The model under review builds one solid part; all positions refer to its coordinate system, in mm. A direction names the side the tool comes from. Give positions to 0.01 mm unless a question says otherwise; leave off trailing zeros. Loops run counter-clockwise (first coordinate to the right, second up) from the corner with the lowest first, then second, coordinate; pieces in that order, holes last. Notation, with made-up numbers: (70.25, -24.75) -> (74.25, -24.75) arc R11 ccw to (74.25, -5.75) -> close; hole circle Ø5 at (61, -1). An arc over 180 degrees is marked (long way). Write each question's results on one line, items separated by ' | '. Start each with the question number.
Q1. Insertion check: pin 1 Ø2 at (x, z) = (14.5, 1) entering from +Y; pin 2 Ø1.2 at (y, z) = (-22, 4) entering from +X; pin 3 Ø2 at (y, z) = (-22.5, 4.5) entering from -X. Each pin has a flat end and moves straight along its axis. Give the tip position at first contact, or say it passes through.
Q2. We need section A-A (y = 35). Write out the cut boundary in (x, z), plus the area to 3 significant figures.
Q3. We need section D-D (y = 2). Write out the cut boundary in (x, z), plus the area to 3 significant figures.
Q4. Wall thickness on L1, parallel to X at y = -15.85, z = 3; L2, parallel to Z at x = 87.5, y = -15.2; L3, parallel to Y at x = -59.5, z = 3.45: over which ranges is each line inside the solid? List them lowest first. Write a range as [from, to].
Q5. We need section C-C (x = -11.5). Write out the cut boundary in (y, z), plus the area to 3 significant figures.
Q6. We need section B-B (z = 3). Give the number of separate pieces and of enclosed holes in the cut face, plus the area to 3 significant figures.
Q7. Mouldability with a two-part tool opening along X and no side actions: class faces 6 (the face through (-90, -22, 3)), 7 (the face through (-20, -22, 3)), 8 (the face through (87, -19.5, 5)) as released by +X, released by -X, zero draft, split by the parting line, or undercut.
Q8. Machinability: for faces 1 (the face through (-84, 11, 3)), 2 (the face through (69.75, 12, 3)), 3 (the face through (-70, -22, 3)), 4 (the face through (61.13, -4.96, 3.04)), 5 (the face through (29.75, 25, 3)), which of the approach directions +Z, -Z, +X, -X, +Y, -Y give a long, thin tool a straight path to every point of the face, cutting with its end or side? Answer none if there is none.
from build123d import *
from build123d.topology import SkipClean

# Parameters (mm, degrees)
SKETCH1_W           = 200
SKETCH1_H           = 45
BOSS_EXTRUDE1_DEPTH = 6
CUT_EXTRUDE1_REACH  = 104.675
SKETCH2_W           = 10
SKETCH2_H           = 3
SKETCH2_W_2         = 50
SKETCH2_W_3         = 25
BOSS_EXTRUDE2_DEPTH = 6
CUT_EXTRUDE2_DEPTH  = 6
CUT_EXTRUDE3_DEPTH  = 6
SKETCH15_R          = 12.5
CUT_EXTRUDE4_DEPTH  = 6
BOSS_EXTRUDE3_DEPTH = 6
SKETCH20_R          = 1.5
CUT_EXTRUDE5_DEPTH  = 111.44568801
SKETCH21_R          = 1.5
CUT_EXTRUDE6_DEPTH  = 117.773284616
SKETCH24_W          = 20
SKETCH24_H          = 6
SKETCH24_W_2        = 25
BOSS_EXTRUDE4_DEPTH = 1
SKETCH25_R          = 6.5
BOSS_EXTRUDE5_DEPTH = 6
SKETCH26_R          = 6.5
CUT_EXTRUDE7_DEPTH  = 111.44568801


with BuildPart() as part:
    # Sketch1 → Boss-Extrude1 (new body)
    with BuildSketch(Plane.XY):
        Rectangle(SKETCH1_W, SKETCH1_H)
    extrude(amount=BOSS_EXTRUDE1_DEPTH)

    # Sketch2 → Cut-Extrude1 (cut, up to next)
    with BuildSketch(Plane.XY.offset(6), mode=Mode.PRIVATE) as cut_extrude1_sk1:
        with Locations((-95, -21)):
            Rectangle(SKETCH2_W, SKETCH2_H)
    cut_extrude1_tool1 = extrude(cut_extrude1_sk1.sketch, amount=-CUT_EXTRUDE1_REACH, mode=Mode.PRIVATE) & part.part
    # Sketch2 → Cut-Extrude1 (cut, up to next)
    with BuildSketch(Plane.XY.offset(6), mode=Mode.PRIVATE) as cut_extrude1_sk2:
        with Locations((-45, -21)):
            Rectangle(SKETCH2_W_2, SKETCH2_H)
    cut_extrude1_tool2 = extrude(cut_extrude1_sk2.sketch, amount=-CUT_EXTRUDE1_REACH, mode=Mode.PRIVATE) & part.part
    # Sketch2 → Cut-Extrude1 (cut, up to next)
    with BuildSketch(Plane.XY.offset(6), mode=Mode.PRIVATE) as cut_extrude1_sk3:
        with Locations((30, -21)):
            Rectangle(SKETCH2_W_2, SKETCH2_H)
    cut_extrude1_tool3 = extrude(cut_extrude1_sk3.sketch, amount=-CUT_EXTRUDE1_REACH, mode=Mode.PRIVATE) & part.part
    # Sketch2 → Cut-Extrude1 (cut, up to next)
    with BuildSketch(Plane.XY.offset(6), mode=Mode.PRIVATE) as cut_extrude1_sk4:
        with Locations((87.5, -21)):
            Rectangle(SKETCH2_W_3, SKETCH2_H)
    cut_extrude1_tool4 = extrude(cut_extrude1_sk4.sketch, amount=-CUT_EXTRUDE1_REACH, mode=Mode.PRIVATE) & part.part
    add(cut_extrude1_tool1.solids().sort_by_distance((-95, -21, 6))[0], mode=Mode.SUBTRACT)
    add(cut_extrude1_tool2.solids().sort_by_distance((-45, -21, 6))[0], mode=Mode.SUBTRACT)
    add(cut_extrude1_tool3.solids().sort_by_distance((30, -21, 6))[0], mode=Mode.SUBTRACT)
    add(cut_extrude1_tool4.solids().sort_by_distance((87.5, -21, 6))[0], mode=Mode.SUBTRACT)

    # Sketch3 → Boss-Extrude2 (add)
    with BuildSketch(Plane.XY.offset(6)):
        with BuildLine():
            Line((-31.5, 42.5), (-31.5, 22.5))
            Line((-31.5, 22.5), (8.5, 22.5))
            Line((8.5, 22.5), (8.5, 42.5))
            Line((8.5, 42.5), (-2, 42.5))
            Line((-2, 42.5), (-2, 37.5))
            Line((-2, 37.5), (-5, 37.5))
            ThreePointArc((-5, 37.5), (-11.5, 31), (-18, 37.5))
            Line((-18, 37.5), (-21, 37.5))
            Line((-21, 37.5), (-21, 42.5))
            Line((-21, 42.5), (-31.5, 42.5))
        make_face()
    extrude(amount=-BOSS_EXTRUDE2_DEPTH)

    # Sketch4 → Cut-Extrude2 (cut)
    with BuildSketch(Plane.XY.offset(6)):
        with BuildLine():
            Line((-53.5, 17.5), (-50.5, 17.5))
            Line((-50.5, 17.5), (-50.5, 22.5))
            Line((-50.5, 22.5), (-69.5, 22.5))
            Line((-69.5, 22.5), (-69.5, 17.5))
            Line((-69.5, 17.5), (-66.5, 17.5))
            ThreePointArc((-66.5, 17.5), (-60, 11), (-53.5, 17.5))
        make_face()
        with BuildLine():
            Line((53, 17.5), (56, 17.5))
            Line((56, 17.5), (56, 22.5))
            Line((56, 22.5), (37, 22.5))
            Line((37, 22.5), (37, 17.5))
            Line((37, 17.5), (40, 17.5))
            ThreePointArc((40, 17.5), (46.5, 11), (53, 17.5))
        make_face()
    extrude(amount=-CUT_EXTRUDE2_DEPTH, mode=Mode.SUBTRACT)

    # Sketch11 → Cut-Extrude3 (cut)
    with BuildSketch(Plane.XY.offset(6)):
        Polygon((-100, -13.5), (-90, -13.5), (-84, -3.107695155), (-84, 22.5), (-100, 22.5), align=None)
        Polygon((100, -13.5), (76.06, -13.5), (69.75, -2.570759404), (69.75, 22.5), (100, 22.5), align=None)
    extrude(amount=-CUT_EXTRUDE3_DEPTH, mode=Mode.SUBTRACT)

    # Sketch15 → Cut-Extrude4 (cut)
    with BuildSketch(Plane.XY.offset(6)):
        with Locations((-34, 0)):
            Circle(SKETCH15_R)
        with Locations((19.75, 0)):
            Circle(SKETCH15_R)
        Polygon((-80, -13.5), (-70, 3.820508076), (-60, 3.820508076), (-69.988315066, -13.5), align=None)
        Polygon((66.06, -13.5), (56.06, 3.820508076), (46.06, 3.820508076), (56.06, -13.5), align=None)
    extrude(amount=-CUT_EXTRUDE4_DEPTH, mode=Mode.SUBTRACT)

    # Sketch19 → Boss-Extrude3 (add)
    with SkipClean():  # the faces are left unmerged after this step: merging them gives an invalid solid
        with BuildSketch(Plane.XY.offset(6)):
            with BuildLine():
                Line((-84, 26.5), (-84, 22.5))
                Line((-84, 22.5), (-69.5, 22.5))
                Line((-69.5, 22.5), (-69.5, 17.5))
                Line((-69.5, 17.5), (-66.5, 17.5))
                ThreePointArc((-66.5, 17.5), (-60, 24), (-53.5, 17.5))
                Line((-53.5, 17.5), (-50.5, 17.5))
                Line((-50.5, 17.5), (-50.5, 22.5))
                Line((-50.5, 22.5), (-31.5, 22.5))
                Line((-31.5, 22.5), (-31.5, 26.5))
                Line((-31.5, 26.5), (-84, 26.5))
            make_face()
            with BuildLine():
                Line((-31.5, 46.5), (-31.5, 42.5))
                Line((-31.5, 42.5), (-21, 42.5))
                Line((-21, 42.5), (-21, 37.5))
                Line((-21, 37.5), (-18, 37.5))
                ThreePointArc((-18, 37.5), (-11.5, 44), (-5, 37.5))
                Line((-5, 37.5), (-2, 37.5))
                Line((-2, 37.5), (-2, 42.5))
                Line((-2, 42.5), (8.5, 42.5))
                Line((8.5, 42.5), (8.5, 46.5))
                Line((8.5, 46.5), (-31.5, 46.5))
            make_face()
            with BuildLine():
                Line((29.75, 26.5), (29.75, 22.5))
                Line((29.75, 22.5), (37, 22.5))
                Line((37, 22.5), (37, 17.5))
                Line((37, 17.5), (40, 17.5))
                ThreePointArc((40, 17.5), (46.5, 24), (53, 17.5))
                Line((53, 17.5), (56, 17.5))
                Line((56, 17.5), (56, 22.5))
                Line((56, 22.5), (69.75, 22.5))
                Line((69.75, 22.5), (69.75, 26.5))
                Line((69.75, 26.5), (29.75, 26.5))
            make_face()
        extrude(amount=-BOSS_EXTRUDE3_DEPTH)

    # Sketch20 → Cut-Extrude5 (cut, through all)
    with SkipClean():  # the faces are left unmerged after this step: merging them gives an invalid solid
        with BuildSketch(Plane(origin=(0, 0, 0), x_dir=(-1, 0, 0), z_dir=(0, 0, -1))):
            with Locations((3, -9.5)):
                Circle(SKETCH20_R)
        extrude(amount=-CUT_EXTRUDE5_DEPTH, mode=Mode.SUBTRACT)

    # Sketch21 → Cut-Extrude6 (cut, through all)
    with SkipClean():  # the faces are left unmerged after this step: merging them gives an invalid solid
        with BuildSketch(Plane(origin=(0, -13.5, 0), x_dir=(1, 0, 0), z_dir=(0, 1, 0))):
            with Locations(Location((87.5, -3, 0), (0, 0, 270))):
                Circle(SKETCH21_R)
            with Locations(Location((-95, -3, 0), (0, 0, 270))):
                Circle(SKETCH21_R)
        extrude(amount=-CUT_EXTRUDE6_DEPTH, mode=Mode.SUBTRACT)

    # Sketch24 → Boss-Extrude4 (add)
    with SkipClean():  # the faces are left unmerged after this step: merging them gives an invalid solid
        with BuildSketch(Plane.XZ.offset(22.5)):
            with Locations((-80, 3)):
                Rectangle(SKETCH24_W, SKETCH24_H)
            with Locations((-7.5, 3)):
                Rectangle(SKETCH24_W_2, SKETCH24_H)
            with Locations((65, 3)):
                Rectangle(SKETCH24_W, SKETCH24_H)
        extrude(amount=BOSS_EXTRUDE4_DEPTH)

    # Sketch25 → Boss-Extrude5 (add)
    with BuildSketch(Plane.XY.offset(6)):
        with Locations((46.5, 17.5)):
            Circle(SKETCH25_R)
        with Locations((-60, 17.5)):
            Circle(SKETCH25_R)
    extrude(amount=-BOSS_EXTRUDE5_DEPTH)

    # Sketch26 → Cut-Extrude7 (cut, through all)
    with BuildSketch(Plane.XY.offset(6)):
        with Locations((55.58, 17.5)):
            Circle(SKETCH26_R)
        with Locations((-60, 17.5)):
            Circle(SKETCH26_R)
    extrude(amount=-CUT_EXTRUDE7_DEPTH, mode=Mode.SUBTRACT)


solid = part.part
Output:
1) pin 1: y = 22.5 | pin 2: x = 75 | pin 3: x = -90
2) outline: (-31.5, 0) -> (-17.5, 0) -> (-17.5, 6) -> (-31.5, 6) -> close; (-5.5, 0) -> (8.5, 0) -> (8.5, 6) -> (-5.5, 6) -> close | area: 168 mm2
3) outline: (-84, 0) -> (-71.05, 0) -> (-71.05, 6) -> (-84, 6) -> close; (-61.05, 0) -> (-46.34, 0) -> (-46.34, 6) -> (-61.05, 6) -> close; (-21.66, 0) -> (7.41, 0) -> (7.41, 6) -> (-21.66, 6) -> close; (32.09, 0) -> (47.11, 0) -> (47.11, 6) -> (32.09, 6) -> close; (57.11, 0) -> (69.75, 0) -> (69.75, 6) -> (57.11, 6) -> close | area: 506 mm2
4) L1: [-100, -96.5], [-93.5, 86], [89, 100] | L2: [0, 1.5], [4.5, 6] | L3: [-19.5, 11.02], [23.98, 26.5]
5) outline: (-23.5, 0) -> (31, 0) -> (31, 6) -> (-23.5, 6) -> close; (44, 0) -> (46.5, 0) -> (46.5, 6) -> (44, 6) -> close | area: 342 mm2
6) separate pieces: 3 | enclosed holes: 8 | area: 6,620 mm2
7) face 6: released by -X | face 7: undercut | face 8: zero draft
8) face 1: +Z, -Z, -X, +Y | face 2: +Z, -Z, +X, +Y | face 3: +Z, -Z, -Y | face 4: +Z, -Z | face 5: +Z, -Z, +Y
